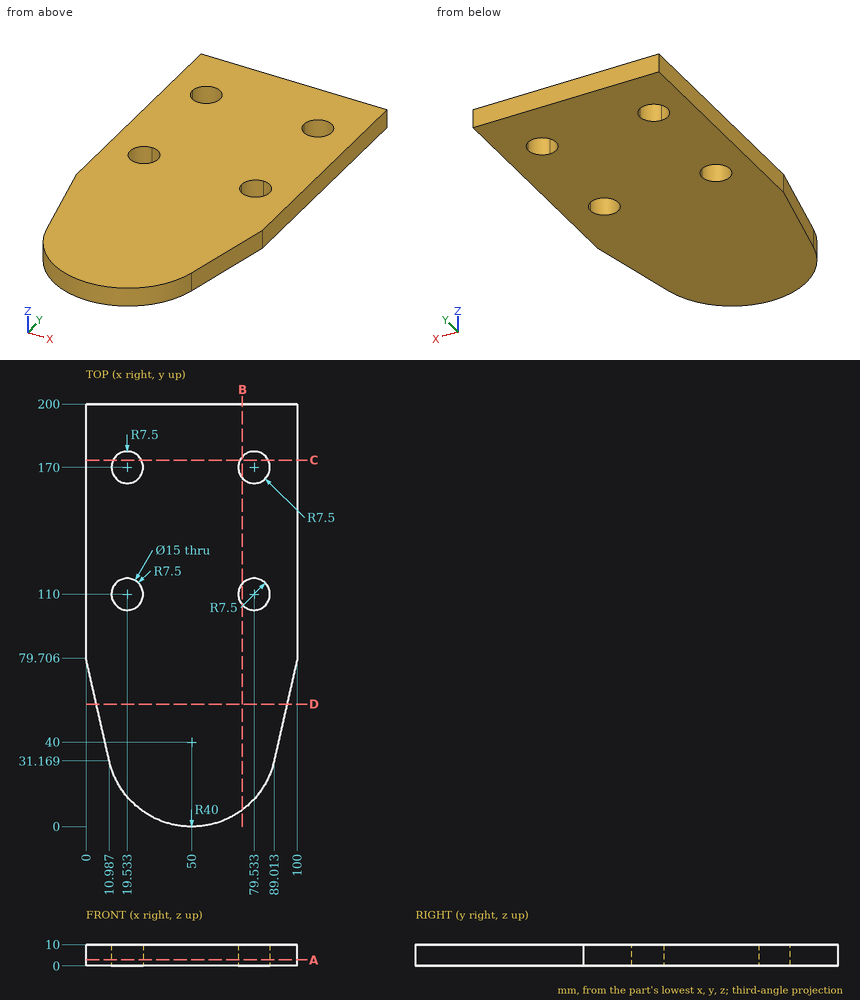
Input: dimensioned drawing with shaded views. Units: mm. Origin: part minimum x, y, z. Round coordinates to 2 decimals unless told otherwise and drop trailing zeros. Order: outer loops, then holes, each group sorted by start corner. A loop starts at its lowest first (then second) coordinate and runs counter-clockwise, first axis right, second up. Notation, with made-up numbers: (51.5, 68) - (78.5, 68) arc R21 ccw to (78.5, 104) - close; hole circle Ø8 at (-15.5, 38). An arc over 180 degrees is marked (long way). Use CSV: the item, a comma, the result in double quotes. Start each with the question number.
Q1. First-contact query: pin 1 (6 mm diameter, centred on y = 65, z = 9, fed in from -X). Flat tip, straight axial feed; report the tip coordinate or a pass-through.
Q2. Material intervals for line 1 along X through (y, z) = (110, 4.5); line 2 along X through (y, z) = (164, 6); line 3 along Y through (x, z) = (24.5, 3.75), sorted ascending. Write a range as from..to.
Q3. Section query B-B (x = 74). Return loops of the section in (y, z), and give its area (3 significant figures).
Q4. Section query A-A (z = 2.75). Return loops of the section in (x, y).
Q5. Section query D-D (y = 58). Return loops of the section in (x, z).
Q6. Section query C-C (y = 173.5). Return loops of the section in (x, z), and give its area (3 significant figures).
Result set:
1,pin 1,"stops at x = 2.65"
2,line 1,"x = 0..12.03, 27.03..72.03, 87.03..100"
2,line 2,"x = 0..15.03, 24.03..75.03, 84.03..100"
2,line 3,"y = 9.18..104.38, 115.62..164.38, 175.62..200"
3,outline,"(8, 0) - (104.94, 0) - (104.94, 10) - (8, 10) - close; (115.06, 0) - (164.94, 0) - (164.94, 10) - (115.06, 10) - close; (175.06, 0) - (200, 0) - (200, 10) - (175.06, 10) - close"
3,area,"1,720 mm2"
4,outline,"(0, 79.71) - (10.99, 31.17) arc R40 ccw to (89.01, 31.17) - (100, 79.71) - (100, 200) - (0, 200) - close; hole circle Ø15 at (19.53, 110); hole circle Ø15 at (19.53, 170); hole circle Ø15 at (79.53, 110); hole circle Ø15 at (79.53, 170)"
5,outline,"(4.91, 0) - (95.09, 0) - (95.09, 10) - (4.91, 10) - close"
6,outline,"(0, 0) - (12.9, 0) - (12.9, 10) - (0, 10) - close; (26.17, 0) - (72.9, 0) - (72.9, 10) - (26.17, 10) - close; (86.17, 0) - (100, 0) - (100, 10) - (86.17, 10) - close"
6,area,"735 mm2"
